For this review, take the finished solid that the model builds, in its own axes (mm). A direction names the side the tool comes from. Coordinates: 2 decimals unless noted, no trailing zeros. Loops run counter-clockwise (first coordinate to the right, second up) from the corner with the lowest first, then second, coordinate; pieces in that order, holes last. Notation, with made-up numbers: (62.5, -13) - (88.5, -13) arc R27 ccw to (88.5, 16) - close; hole circle Ø6 at (39.5, 9). An arc over 180 degrees is marked (long way). One line per item, written item: value. Start each with the question number.
1. To check wall thickness, follow line 1 (X direction, y = 3.25, z = 4); line 2 (X direction, y = -0.5, z = -8.75); line 3 (Z direction, x = 43, y = 6). State the ranges of each line that lie inside material, in increasing order. Write a range as from..to.
2. For faces 1 (the face through (24, 0, 5)), 2 (the face through (109, 0, 0)), 3 (the face through (30.409, -8.428, -1.107)), list the 3-axis set-ups (+Z, -Z, +X, -X, +Y, -Y) from which the entire face can be reached by the end or side of a thin tool; tool diameter is ignored.
3. The part is to be moulded in two halves that separate along X. For faces 4 (the face through (2.72, -4.88, 1.08)), 5 (the face through (0, 0, 0)), 6 (the face through (15, 2.5, 5)), say which applies: released by +X, released by -X, zero draft, split by the parting line, or undercut.
4. Insertion check: pin 1 (8.5 mm diameter, centred on y = 1, z = -7, fed in from -X); pin 2 (3 mm diameter, centred on y = 6.5, z = -5, fed in from -X); pin 3 (6.5 mm diameter, centred on x = 76.5, y = 0, fed in from +Z); pin 4 (4 mm diameter, centred on x = 18.5, y = 0, fed in from +Z). Each pin has a flat end and moves straight along its axis. Give the tip position at first contact, or say it passes through.
5. Take a section at A-A, the plane x = 66. State the section outline as (y, z) points, and give its area (3 significant figures).
6. Take a section at B-B, the plane x = 52. State the section outline as (y, z) points.
```python
from build123d import *

# Parameters (mm, degrees)
SKETCH1_R           = 5
BOSS_EXTRUDE1_DEPTH = 5
SKETCH2_R           = 7
BOSS_EXTRUDE2_DEPTH = 19
SKETCH3_R           = 8.5
BOSS_EXTRUDE3_DEPTH = 13
SKETCH4_R           = 10
BOSS_EXTRUDE4_DEPTH = 19
SKETCH5_R           = 14.5
BOSS_EXTRUDE5_DEPTH = 8
SKETCH6_R           = 11.5
BOSS_EXTRUDE6_DEPTH = 23
SKETCH7_R           = 8.5
BOSS_EXTRUDE7_DEPTH = 22
CHAMFER1_SIZE       = 0.5
CUT_EXTRUDE2_START  = 7
CUT_EXTRUDE2_DEPTH  = 3.5
CUT_EXTRUDE3_START  = 11.5
CUT_EXTRUDE3_DEPTH  = 6.5
FILLET1_R           = 2


with BuildPart() as part:
    # Sketch1 → Boss-Extrude1 (new body)
    with BuildSketch(Plane(origin=(0, 0, 0), x_dir=(0, 0, -1), z_dir=(1, 0, 0))):
        Circle(SKETCH1_R)
    extrude(amount=BOSS_EXTRUDE1_DEPTH)

    # Sketch2 → Boss-Extrude2 (add)
    with BuildSketch(Plane(origin=(5, 0, 0), x_dir=(0, 0, -1), z_dir=(1, 0, 0))):
        Circle(SKETCH2_R)
    extrude(amount=BOSS_EXTRUDE2_DEPTH)

    # Sketch3 → Boss-Extrude3 (add)
    with BuildSketch(Plane(origin=(24, 0, 0), x_dir=(0, 0, -1), z_dir=(1, 0, 0))):
        with Locations(Location((0, 0, 0), (0, 0, 180))):
            Circle(SKETCH3_R)
    extrude(amount=BOSS_EXTRUDE3_DEPTH)

    # Sketch4 → Boss-Extrude4 (add)
    with BuildSketch(Plane(origin=(37, 0, 0), x_dir=(0, 0, -1), z_dir=(1, 0, 0))):
        Circle(SKETCH4_R)
    extrude(amount=BOSS_EXTRUDE4_DEPTH)

    # Sketch5 → Boss-Extrude5 (add)
    with BuildSketch(Plane(origin=(56, 0, 0), x_dir=(0, 0, -1), z_dir=(1, 0, 0))):
        Circle(SKETCH5_R)
    extrude(amount=BOSS_EXTRUDE5_DEPTH)

    # Sketch6 → Boss-Extrude6 (add)
    with BuildSketch(Plane(origin=(64, 0, 0), x_dir=(0, 0, -1), z_dir=(1, 0, 0))):
        Circle(SKETCH6_R)
    extrude(amount=BOSS_EXTRUDE6_DEPTH)

    # Sketch7 → Boss-Extrude7 (add)
    with BuildSketch(Plane(origin=(87, 0, 0), x_dir=(0, 0, -1), z_dir=(1, 0, 0))):
        with Locations(Location((0, 0, 0), (0, 0, 180))):
            Circle(SKETCH7_R)
    extrude(amount=BOSS_EXTRUDE7_DEPTH)

    # Chamfer1
    chamfer1_edges = [part.edges().sort_by_distance(p)[0] for p in [
        (37, 0, 10),
        (56, 0, 14.5),
        (0, 0, 5),
        (64, 0, 14.5),
        (87, 0, 11.5),
        (109, 0, -8.5),
        (5, 0, 7),
    ]]
    chamfer(chamfer1_edges, length=CHAMFER1_SIZE)

    # Sketch8 → Cut-Extrude2 (cut)
    with BuildSketch(Plane.XY.offset(CUT_EXTRUDE2_START)):
        with BuildLine():
            Line((8.5, 2.5), (21.5, 2.5))
            ThreePointArc((21.5, 2.5), (24, 0), (21.5, -2.5))
            Line((21.5, -2.5), (8.5, -2.5))
            ThreePointArc((8.5, -2.5), (6, 0), (8.5, 2.5))
        make_face()
    extrude(amount=-CUT_EXTRUDE2_DEPTH, mode=Mode.SUBTRACT)

    # Sketch9 → Cut-Extrude3 (cut)
    with BuildSketch(Plane.XY.offset(CUT_EXTRUDE3_START)):
        with BuildLine():
            Line((71.5, 3), (79.5, 3))
            ThreePointArc((79.5, 3), (82.5, 0), (79.5, -3))
            Line((79.5, -3), (71.5, -3))
            ThreePointArc((71.5, -3), (68.5, 0), (71.5, 3))
        make_face()
    extrude(amount=-CUT_EXTRUDE3_DEPTH, mode=Mode.SUBTRACT)

    # Fillet1
    fillet1_edges = [part.edges().sort_by_distance(p)[0] for p in [
        (56, 0, 10),
    ]]
    fillet(fillet1_edges, radius=FILLET1_R)


solid = part.part
```
Solutions:
1. line 1: 5..109
1. line 2: 37..87
1. line 3: -8..8
2. face 1: +Z
2. face 2: +Z, -Z, +X, +Y, -Y
2. face 3: -X
3. face 4: zero draft
3. face 5: released by -X
3. face 6: undercut
4. pin 1: x = 0
4. pin 2: x = 5.2
4. pin 3: z = 11.1
4. pin 4: z = 3.5
5. outline: circle Ø23 at (0, 0)
5. area: 415 mm2
6. outline: circle Ø20 at (0, 0)
